```python
from build123d import *

# Parameters (mm, degrees)
EXTRUDE_1_DEPTH = 585


with BuildPart() as part:
    # 草图1 → 拉伸1 (new body)
    with BuildSketch(Plane.XY):
        with BuildLine():
            Line((-1.661470687, 4.25), (1.661470687, 4.25))
            ThreePointArc((1.661470687, 4.25), (3.001099397, 3.934286669), (4.058769011, 3.053596614))
            ThreePointArc((4.058769011, 3.053596614), (5.079178887, 0), (4.058769011, -3.053596614))
            ThreePointArc((4.058769011, -3.053596614), (3.001099397, -3.934286669), (1.661470687, -4.25))
            Line((1.661470687, -4.25), (-1.661470687, -4.25))
            ThreePointArc((-1.661470687, -4.25), (-3.001099397, -3.934286669), (-4.058769011, -3.053596614))
            ThreePointArc((-4.058769011, -3.053596614), (-5.079178887, 0), (-4.058769011, 3.053596614))
            ThreePointArc((-4.058769011, 3.053596614), (-3.001099397, 3.934286669), (-1.661470687, 4.25))
        make_face()
    extrude(amount=EXTRUDE_1_DEPTH)


solid = part.part
```
Check sheet for the modelled part. Datum: model origin and axes. Units: mm. Round coordinates to 2 decimals unless told otherwise and drop trailing zeros. Write each loop counter-clockwise with the first axis right and the second up, starting at its lowest first coordinate (ties: lowest second). Pieces come first, ordered by that corner, then holes. Notation, with made-up numbers: (62, 24) -> (88, 24) arc R27 ccw to (88, 43) -> close; hole circle Ø9 at (18.25, 78.25). An arc over 180 degrees is marked (long way). Put each result on its own line as item: value.
(1) Sectioned sample at B-B (y = -1.5). Enter the section's corners in (x, z), plus the area to 3 significant figures.
Values found:
outline: (-4.85, 0) -> (4.85, 0) -> (4.85, 585) -> (-4.85, 585) -> close
area: 5,680 mm^2
(2) Material ranges on line 1 (X direction, y = -0.5, z = 61); line 2 (X direction, y = -1, z = 371.5); line 3 (Y direction, x = -2, z = 555), recorded low to high.
Values found:
line 1: x = -5.05 to 5.05
line 2: x = -4.98 to 4.98
line 3: y = -4.23 to 4.23
(3) Go/stop test with a flat-tipped pin: pin 1 Ø5 at (y, z) = (3.5, 131.5) entering from +X. Record where the tip stops, or that it passes through.
Values found:
pin 1: stops at x = 4.98
(4) Sectioned sample at A-A (z = 255.5). Enter the section's corners in (x, y).
Values found:
outline: (-4.06, -3.05) arc R3 ccw to (-1.66, -4.25) -> (1.66, -4.25) arc R3 ccw to (4.06, -3.05) arc R5.08 ccw to (4.06, 3.05) arc R3 ccw to (1.66, 4.25) -> (-1.66, 4.25) arc R3 ccw to (-4.06, 3.05) arc R5.08 ccw to start
